For this review, take the finished solid that the model builds, in its own axes (mm). A direction names the side the tool comes from. Round coordinates to 2 decimals unless told otherwise and drop trailing zeros. Write each loop counter-clockwise with the first axis right and the second up, starting at its lowest first coordinate (ties: lowest second). Pieces come first, ordered by that corner, then holes. Notation, with made-up numbers: (-12, 26) -> (43, 26) arc R22 ccw to (43, 45) -> close; hole circle Ø3 at (56, -27). An arc over 180 degrees is marked (long way). Answer in a Markdown table with one row per item.
from build123d import *

# Parameters (mm, degrees)
SKETCH1_R                = 2.5
F_20_X_20_X_R1_5_1_DEPTH = 260


with BuildPart() as part:
    # Sketch1 → 工业铝型材 20 X 20 X R1.5(1) (new body)
    with BuildSketch(Plane.YZ):
        with BuildLine():
            Line((-3.6, 10), (-3.6, 9.5))
            Line((-3.6, 9.5), (-3.1, 9.5))
            Line((-3.1, 9.5), (-3.1, 8.5))
            Line((-3.1, 8.5), (-5.5, 8.5))
            Line((-5.5, 8.5), (-5.5, 6.65))
            Line((-5.5, 6.65), (-2.75, 3.9))
            Line((-2.75, 3.9), (2.75, 3.9))
            Line((2.75, 3.9), (5.5, 6.65))
            Line((5.5, 6.65), (5.5, 8.5))
            Line((5.5, 8.5), (3.1, 8.5))
            Line((3.1, 8.5), (3.1, 9.5))
            Line((3.1, 9.5), (3.6, 9.5))
            Line((3.6, 9.5), (3.6, 10))
            Line((3.6, 10), (8.5, 10))
            ThreePointArc((8.5, 10), (9.560660172, 9.560660172), (10, 8.5))
            Line((10, 8.5), (10, 3.6))
            Line((10, 3.6), (9.5, 3.6))
            Line((9.5, 3.6), (9.5, 3.1))
            Line((9.5, 3.1), (8.5, 3.1))
            Line((8.5, 3.1), (8.5, 5.5))
            Line((8.5, 5.5), (6.65, 5.5))
            Line((6.65, 5.5), (3.9, 2.75))
            Line((3.9, 2.75), (3.9, -2.75))
            Line((3.9, -2.75), (6.65, -5.5))
            Line((6.65, -5.5), (8.5, -5.5))
            Line((8.5, -5.5), (8.5, -3.1))
            Line((8.5, -3.1), (9.5, -3.1))
            Line((9.5, -3.1), (9.5, -3.6))
            Line((9.5, -3.6), (10, -3.6))
            Line((10, -3.6), (10, -8.5))
            ThreePointArc((10, -8.5), (9.560660172, -9.560660172), (8.5, -10))
            Line((8.5, -10), (3.6, -10))
            Line((3.6, -10), (3.6, -9.5))
            Line((3.6, -9.5), (3.1, -9.5))
            Line((3.1, -9.5), (3.1, -8.5))
            Line((3.1, -8.5), (5.5, -8.5))
            Line((5.5, -8.5), (5.5, -6.65))
            Line((5.5, -6.65), (2.75, -3.9))
            Line((2.75, -3.9), (-2.75, -3.9))
            Line((-2.75, -3.9), (-5.5, -6.65))
            Line((-5.5, -6.65), (-5.5, -8.5))
            Line((-5.5, -8.5), (-3.1, -8.5))
            Line((-3.1, -8.5), (-3.1, -9.5))
            Line((-3.1, -9.5), (-3.6, -9.5))
            Line((-3.6, -9.5), (-3.6, -10))
            Line((-3.6, -10), (-8.5, -10))
            ThreePointArc((-8.5, -10), (-9.560660172, -9.560660172), (-10, -8.5))
            Line((-10, -8.5), (-10, -3.6))
            Line((-10, -3.6), (-9.5, -3.6))
            Line((-9.5, -3.6), (-9.5, -3.1))
            Line((-9.5, -3.1), (-8.5, -3.1))
            Line((-8.5, -3.1), (-8.5, -5.5))
            Line((-8.5, -5.5), (-6.65, -5.5))
            Line((-6.65, -5.5), (-3.9, -2.75))
            Line((-3.9, -2.75), (-3.9, 2.75))
            Line((-3.9, 2.75), (-6.65, 5.5))
            Line((-6.65, 5.5), (-8.5, 5.5))
            Line((-8.5, 5.5), (-8.5, 3.1))
            Line((-8.5, 3.1), (-9.5, 3.1))
            Line((-9.5, 3.1), (-9.5, 3.6))
            Line((-9.5, 3.6), (-10, 3.6))
            Line((-10, 3.6), (-10, 8.5))
            ThreePointArc((-10, 8.5), (-9.560660172, 9.560660172), (-8.5, 10))
            Line((-8.5, 10), (-3.6, 10))
        make_face()
        Circle(SKETCH1_R, mode=Mode.SUBTRACT)
    extrude(amount=F_20_X_20_X_R1_5_1_DEPTH)


solid = part.part
1) For faces 5 (the flat face through (128, 10, -6)), 6 (the flat face through (128, -3.9, 0)), 7 (the flat face through (128, 0, -3.9)), list the 3-axis set-ups (+Z, -Z, +X, -X, +Y, -Y) from which the entire face can be reached by the end or side of a thin tool; tool diameter is ignored.
Solved:
| item | result |
|---|---|
| face 5 | +Z, -Z, +X, -X, +Y |
| face 6 | +X, -X, -Y |
| face 7 | -Z, +X, -X |
2) Clearance check with flat-ended pins moving along their axes: pin 1 Ø3 at (x, z) = (119, 0) entering from -Y; pin 2 Ø1 at (x, y) = (85.5, 1) entering from -Z; pin 3 Ø1.5 at (y, z) = (7, 1) entering from +X; pin 4 Ø3 at (x, z) = (228, -1.5) entering from -Y. State where each tip first meets the part, or that it passes through.
Solved:
| item | result |
|---|---|
| pin 1 | y = -3.9 |
| pin 2 | z = -3.9 |
| pin 3 | through |
| pin 4 | y = -4.15 |
3) For line 1 (Z direction, x = 147, y = 0); line 2 (Z direction, x = 121.5, y = -6.75); line 3 (Z direction, x = 53, y = -3.5), list the stretches that pass through material, from the lowest coordinate up. Write a range as [from, to].
Solved:
| item | result |
|---|---|
| line 1 | [-3.9, -2.5], [2.5, 3.9] |
| line 2 | [-10, -5.5], [5.5, 10] |
| line 3 | [-9.5, -8.5], [-4.65, 4.65], [8.5, 9.5] |
4) Consider section A-A on z = 0. State the section outline as (x, y) points, then the cut area to 3 significant figures.
Solved:
| item | result |
|---|---|
| outline | (0, -3.9) -> (260, -3.9) -> (260, -2.5) -> (0, -2.5) -> close; (0, 2.5) -> (260, 2.5) -> (260, 3.9) -> (0, 3.9) -> close |
| area | 728 mm² |
5) Mouldability with a two-part tool opening along Z and no side actions: class faces 1 (the flat face through (128, 10, 6)), 2 (the flat face through (128, 3.9, 0)), 3 (the flat face through (128, 0, 3.9)), 4 (the cylindrical face through (128.18, -0.54, -2.44)) as pulls with the +Z half, pulls with the -Z half, needs draft (parallel to the pull), parting line crosses it, or undercut.
Solved:
| item | result |
|---|---|
| face 1 | needs draft |
| face 2 | undercut |
| face 3 | pulls with the +Z half |
| face 4 | undercut |
